Design review of the part shown in the three views and the two pictorial views. Dimensions are in mm from the part's minimum x, y and z. Coordinates: 2 decimals unless noted, no trailing zeros. Order: outer loops, then holes, each group sorted by start corner. A loop starts at its lowest first (then second) coordinate and runs counter-clockwise, first axis right, second up. Notation, with made-up numbers: (-34, 6.5) - (21, 6.5) arc R18 ccw to (21, 11.5) - close; hole circle Ø9 at (-21, 17.25). An arc over 180 degrees is marked (long way). One line per item, written item: value. Start each with the question number.
(1) Consider section B-B on y = 65. Write out the cut boundary in (x, z).
(2) To check wall thickness, follow line 1 along Y through (x, z) = (18.5, 409.5); line 2 along Z through (x, y) = (10.25, 65); line 3 along X through (y, z) = (94, 750). State the ranges of each line that lie inside material, in increasing order.
(3) Consider section C-C on x = 32. Write out the cut boundary in (y, z), then the cut area to 4 significant figures.
(4) Clearance check with flat-ended pins moving along their axes: pin 1 (2 mm diameter, centred on y = 87.5, z = 450.5, fed in from +X); pin 2 (5 mm diameter, centred on x = 26, z = 195, fed in from -Y). State where each tip first meets the part, or that it passes through.
(5) Consider section A-A on z = 370. Write out the cut boundary in (x, y).
(6) Consider section D-D on z = 707. Write out the cut boundary in (x, y).
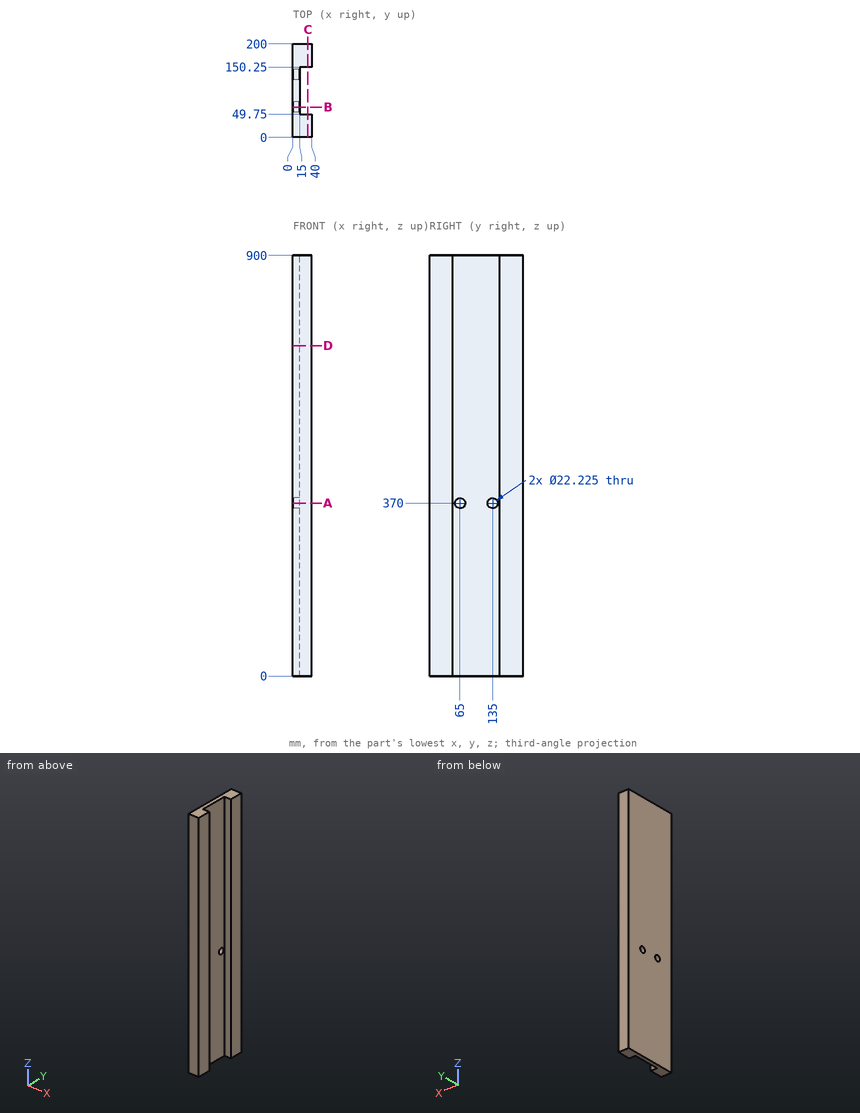
Geometry check:
1. outline: (0, 0) - (15, 0) - (15, 358.89) - (0, 358.89) - close; (0, 381.11) - (15, 381.11) - (15, 900) - (0, 900) - close
2. line 1: y = 0 to 49.75, 150.25 to 200
2. line 2: z = 0 to 358.89, 381.11 to 900
2. line 3: x = 0 to 15
3. outline: (0, 0) - (49.75, 0) - (49.75, 900) - (0, 900) - close; (150.25, 0) - (200, 0) - (200, 900) - (150.25, 900) - close
3. area: 89,550 mm^2
4. pin 1: stops at x = 15
4. pin 2: stops at y = 0
5. outline: (0, 0) - (40, 0) - (40, 49.75) - (15, 49.75) - (15, 53.89) - (0, 53.89) - close; (0, 76.11) - (15, 76.11) - (15, 123.89) - (0, 123.89) - close; (0, 146.11) - (15, 146.11) - (15, 150.25) - (40, 150.25) - (40, 200) - (0, 200) - close
6. outline: (0, 0) - (40, 0) - (40, 49.75) - (15, 49.75) - (15, 150.25) - (40, 150.25) - (40, 200) - (0, 200) - close
